```python
from build123d import *

# Parameters (mm, degrees)
SKETCH_1_W          = 265
SKETCH_1_H          = 260
EXTRUDE_1_DEPTH     = 15
HOLE_WIZARD_M10_1_D = 8.5
SKETCH_4_W          = 105
SKETCH_4_H          = 85
CUT_EXTRUDE_1_DEPTH = 187.229025665
FILLET_1_R          = 10
SKETCH_5_R          = 35
CUT_EXTRUDE_2_DEPTH = 187.229025665
CHAMFER_2_SIZE      = 1
CHAMFER_1_SIZE      = 30
CHAMFER_3_SIZE      = 10


with BuildPart() as part:
    # 草图1 → 凸台-拉伸1 (new body)
    with BuildSketch(Plane.XY):
        Rectangle(SKETCH_1_W, SKETCH_1_H)
    extrude(amount=EXTRUDE_1_DEPTH)

    # M10 螺纹孔1 (through all)
    with Locations(Plane(origin=(0, 0, 0), x_dir=(-1, 0, 0), z_dir=(0, 0, -1))):
        with Locations((-80, 115), (-115, 70), (-115, -70), (-80, -115), (80, -115), (115, -70), (115, 70), (80, 115)):
            Hole(HOLE_WIZARD_M10_1_D / 2)

    # 草图4 → 切除-拉伸1 (cut, through all)
    with BuildSketch(Plane(origin=(0, 0, 0), x_dir=(-1, 0, 0), z_dir=(0, 0, -1))):
        with Locations((0, -87.5)):
            Rectangle(SKETCH_4_W, SKETCH_4_H)
    extrude(amount=-CUT_EXTRUDE_1_DEPTH, mode=Mode.SUBTRACT)

    # 圆角1
    fillet_1_edges = [part.edges().sort_by_distance(p)[0] for p in [
        (52.5, -45, 7.5),
        (-52.5, -45, 7.5),
    ]]
    fillet(fillet_1_edges, radius=FILLET_1_R)

    # 草图5 → 切除-拉伸2 (cut, through all)
    with BuildSketch(Plane(origin=(0, 0, 0), x_dir=(-1, 0, 0), z_dir=(0, 0, -1))):
        Circle(SKETCH_5_R)
    extrude(amount=-CUT_EXTRUDE_2_DEPTH, mode=Mode.SUBTRACT)

    # 倒角2
    chamfer_2_edges = [part.edges().sort_by_distance(p)[0] for p in [
        (35, 0, 15),
        (35, 0, 0),
    ]]
    chamfer(chamfer_2_edges, length=CHAMFER_2_SIZE)

    # 倒角1
    chamfer_1_edges = [part.edges().sort_by_distance(p)[0] for p in [
        (132.5, -130, 7.5),
        (-132.5, -130, 7.5),
        (-132.5, 130, 7.5),
        (132.5, 130, 7.5),
    ]]
    chamfer(chamfer_1_edges, length=CHAMFER_1_SIZE)

    # 倒角3
    chamfer_3_edges = [part.edges().sort_by_distance(p)[0] for p in [
        (52.5, -130, 7.5),
        (-52.5, -130, 7.5),
    ]]
    chamfer(chamfer_3_edges, length=CHAMFER_3_SIZE)


solid = part.part
```
Model file for the job. Use its own axes, mm. A direction names the side the tool comes from. Give positions to 0.01 mm unless a question says otherwise; leave off trailing zeros. Loops run counter-clockwise (first coordinate to the right, second up) from the corner with the lowest first, then second, coordinate; pieces in that order, holes last. Notation, with made-up numbers: (66, 1.5) -> (109, 1.5) arc R23 ccw to (109, 13.5) -> close; hole circle Ø8 at (54, 13). An arc over 180 degrees is marked (long way). Use CSV: the item, a comma, the result in double quotes. Start each with the question number.
1) Tool access for faces 1 (the flat face through (52.5, -88, 7)), 2 (the flat face through (117.7, -114.8, 7.4)): list every direction of +Z, -Z, +X, -X, +Y, -Y with a clear straight run to the whole face (end or side of a thin tool).
2) Wall check: line 1 (Y direction, x = 80, z = 8.5); line 2 (X direction, y = -65, z = 5.5); line 3 (Y direction, x = -115, z = 12). Give the ranges that are in metal, low to high.
3) Slice it at B-B on x = -80. Give the cut face in (y, z).
4) Slice it at A-A on x = 0. Give the cut face in (y, z), plus the area to 3 significant figures.
5) Slice it at C-C on y = 115. Give the cut face in (x, z), plus the area to 3 significant figures.
6) Mould opens along Y. For faces 3 (the cylindrical face through (82.285, -111.416, 7.605)), 4 (the flat face through (-117.7, 114.8, 7.4)), 5 (the flat face through (28, 31, 0)) say: released by +Y, released by -Y, zero draft, split by the parting line, or undercut.
7) Flat gauge pins, fed straight in: pin 1 Ø7.5 at (x, z) = (-7, 10.5) entering from -Y; pin 2 Ø7 at (x, y) = (80, -115) entering from +Z. Where does each tip first touch, or does it go through?
8) Slice it at D-D on z = 6.75. Give the number of separate pieces and of enclosed holes in the cut face, plus the area to 3 significant figures.
Computed values:
1,face 1,"+Z, -Z, -Y"
1,face 2,"+Z, -Z, +X, -Y"
2,line 1,"y = -130 to -119.25, -110.75 to 110.75, 119.25 to 130"
2,line 2,"x = -132.5 to -52.5, 52.5 to 132.5"
2,line 3,"y = -117.5 to -74.25, -65.75 to 65.75, 74.25 to 117.5"
3,outline,"(-130, 0) -> (-119.25, 0) -> (-119.25, 15) -> (-130, 15) -> close; (-110.75, 0) -> (110.75, 0) -> (110.75, 15) -> (-110.75, 15) -> close; (119.25, 0) -> (130, 0) -> (130, 15) -> (119.25, 15) -> close"
4,outline,"(-45, 0) -> (-36, 0) -> (-35, 1) -> (-35, 14) -> (-36, 15) -> (-45, 15) -> close; (35, 1) -> (36, 0) -> (130, 0) -> (130, 15) -> (36, 15) -> (35, 14) -> close"
4,area,"1,570 mm^2"
5,outline,"(-117.5, 0) -> (-84.25, 0) -> (-84.25, 15) -> (-117.5, 15) -> close; (-75.75, 0) -> (75.75, 0) -> (75.75, 15) -> (-75.75, 15) -> close; (84.25, 0) -> (117.5, 0) -> (117.5, 15) -> (84.25, 15) -> close"
5,area,"3,270 mm^2"
6,face 3,"undercut"
6,face 4,"released by +Y"
6,face 5,"zero draft"
7,pin 1,"stops at y = -45"
7,pin 2,"passes through"
8,separate pieces,"1"
8,enclosed holes,"9"
8,area,"53,800 mm^2"
